from build123d import *

# Parameters (mm, degrees)
CHAMFER1_SIZE = 1
CHAMFER2_SIZE = 0.5
SKETCH2_R     = 1


with BuildPart() as part:
    # Sketch1 → Revolve1 (revolve)
    with BuildSketch(Plane.XY, mode=Mode.PRIVATE) as revolve1_sk:
        Polygon((30, 8.5), (0, 8.5), (0, 13.5), (4, 13.5), (4, 11), (30, 11), align=None)
    revolve(revolve1_sk.sketch.rotate(Axis((0, 0, 0), (1, 0, 0)), 90), axis=Axis((0, 0, 0), (1, 0, 0)))

    # Chamfer1
    chamfer1_edges = [part.edges().sort_by_distance(p)[0] for p in [
        (0, 0, -13.5),
    ]]
    chamfer(chamfer1_edges, length=CHAMFER1_SIZE)

    # Chamfer2
    chamfer2_edges = [part.edges().sort_by_distance(p)[0] for p in [
        (30, 0, -11),
        (4, 0, -13.5),
        (0, 0, -8.5),
        (30, 0, -8.5),
    ]]
    chamfer(chamfer2_edges, length=CHAMFER2_SIZE)

    # Sketch2 → Cut-Revolve1 (revolve, cut)
    with BuildSketch(Plane(origin=(0, 0, 0), x_dir=(1, 0, 0), z_dir=(0, 1, 0))):
        with Locations((32, 11)):
            Circle(SKETCH2_R)
        with Locations((17, 11)):
            Circle(SKETCH2_R)
        Polygon((4, 11), (4, 10), (5.8, 10), (6, 11), align=None)
    revolve(axis=Axis((29.5, 0, 0), (-1, 0, 0)), mode=Mode.SUBTRACT)


solid = part.part
Could you check a few things on this model? Use its own coordinates, in mm. A direction names the side the tool comes from. Coordinates: 2 decimals unless noted, no trailing zeros. Order: outer loops, then holes, each group sorted by start corner. A loop starts at its lowest first (then second) coordinate and runs counter-clockwise, first axis right, second up.
Q1. Suppose I cut it at C-C on x = 23.5. Please give me the cut outline in (y, z), and give its area (3 significant figures).
Q2. Will these pins go through, and if not, where does the flat tip stop? pin 1 (12 mm diameter, centred on x = 24.5, z = -2, fed in from -Y); pin 2 (10 mm diameter, centred on y = -10.5, z = 6.5, fed in from -X); pin 3 (5 mm diameter, centred on x = 3, y = -4.5, fed in from -Z); pin 4 (1 mm diameter, centred on x = 25.5, z = -3.5, fed in from -Y).
Q3. Which directions (+Z, -Z, +X, -X, +Y, -Y) give clear straight access to the entire face, cutting with the end or side of a thin tool? Please do faces 5 (the cylindrical face through (2.27, 13.18, -2.93)), 6 (the cylindrical face through (23.83, 10.74, -2.38)).
Q4. Please list where these lines run through material, in increasing order: L1, parallel to Z at x = 14.25, y = 0.25; L2, parallel to X at y = -8, z = 10.25.
Q5. Thinking about a two-plate mould opening in X: for faces 1 (the cylindrical face through (11.07, 10.74, -2.38)), 2 (the flat face through (4, 8, 7)), 3 (the flat face through (30, -5, 8)), 4 (the cylindrical face through (4.91, 9.76, 2.17)), which applies, released by +X, released by -X, zero draft, split by the parting line, or undercut?
Answer:
1. outline: circle Ø22 at (0, 0); hole circle Ø17 at (0, 0)
1. area: 153 mm2
2. pin 1: stops at y = -11
2. pin 2: stops at x = 0
2. pin 3: stops at z = -13.35
2. pin 4: stops at y = -10.58
3. face 5: +X, -X
3. face 6: +X
4. L1: z = -11 to -8.5, 8.5 to 11
4. L2: x = 0.5 to 4
5. face 1: zero draft
5. face 2: undercut
5. face 3: released by +X
5. face 4: undercut
